Verification items for the finished model (mm, model axes). A direction names the side the tool comes from. Round coordinates to 2 decimals unless told otherwise and drop trailing zeros. Order: outer loops, then holes, each group sorted by start corner. A loop starts at its lowest first (then second) coordinate and runs counter-clockwise, first axis right, second up. Notation, with made-up numbers: (82.5, 20.5) -> (135.5, 20.5) arc R16 ccw to (135.5, 51.5) -> close; hole circle Ø7 at (0, -6.5). An arc over 180 degrees is marked (long way). Answer in a Markdown table with one row per item. Add a question column.
```python
from build123d import *

# Parameters (mm, degrees)
HEX_HEAD_15AF_DEPTH = 8


with BuildPart() as part:
    # Hex Head Profile → Hex Head 15AF (new body)
    with BuildSketch(Plane(origin=(0, 0, 0), x_dir=(1, 0, 0), z_dir=(0, 1, 0))):
        Polygon((8.660254038, 0), (4.330127019, 7.5), (-4.330127019, 7.5), (-8.660254038, 0), (-4.330127019, -7.5), (4.330127019, -7.5), align=None)
    extrude(amount=HEX_HEAD_15AF_DEPTH)

    # Shank Profile → Shank with Cone Point (revolve)
    with BuildSketch(Plane.XY, mode=Mode.PRIVATE) as shank_with_cone_point_sk:
        Polygon((0, 8), (0, 23.886751346), (5, 21), (5, 8), align=None)
    revolve(shank_with_cone_point_sk.sketch.rotate(Axis((0, 23.886751346, 0), (0, 1, 0)), 90), axis=Axis((0, 23.886751346, 0), (0, 1, 0)))

    # Head Chamfer Profile → Head Chamfer Cut (revolve, cut)
    with BuildSketch(Plane.XY, mode=Mode.PRIVATE) as head_chamfer_cut_sk:
        with BuildLine():
            Line((8.660254038, 0), (6.660254038, 0))
            ThreePointArc((6.660254038, 0), (8.0744676, 0.585786438), (8.660254038, 2))
            Line((8.660254038, 2), (8.660254038, 0))
        make_face()
    revolve(head_chamfer_cut_sk.sketch.rotate(Axis((0, 0, 0), (0, 1, 0)), 90), axis=Axis((0, 0, 0), (0, 1, 0)), mode=Mode.SUBTRACT)


solid = part.part
```
1) Cross-section at C-C, the plane y = 21.5. Record the boundary of the cut face in (x, z).
2) Tool access check on faces 1 (the face through (6.526, 4.038, -3.698)), 2 (the face through (2, 8, -5)). Record the directions out of +Z, -Z, +X, -X, +Y, -Y that give a thin tool (end or side, any length) a straight path to the whole face; none if there is none.
3) Cross-section at B-B, the plane y = 17.75. Record the boundary of the cut face in (x, z).
4) Cross-section at A-A, the plane y = 3.75. Record the boundary of the cut face in (x, z).
5) Depth check by flat-ended pin: P1, Ø6, axis at y = 13.5, z = -2, coming from the +X side; P2, Ø4, axis at x = 6.5, z = 0, coming from the +Y side; P3, Ø4, axis at x = 4.5, y = 16, coming from the -Z side. Enter the tip coordinate at first touch or a pass-through.
6) Thickness scan on L1, parallel to X at y = 15.5, z = -0.25; L2, parallel to Y at x = 1.5, z = -6.25; L3, parallel to Y at x = 4.25, z = 1.5. Record the ranges inside material, lowest first. Write a range as [from, to].
Results below:
| question | item | result |
|---|---|---|
| 1 | outline | circle Ø8.27 at (0, 0) |
| 2 | face 1 | -Z, +X, +Y, -Y |
| 2 | face 2 | +Y |
| 3 | outline | circle Ø10 at (0, 0) |
| 4 | outline | (-8.66, 0) -> (-4.33, -7.5) -> (4.33, -7.5) -> (8.66, 0) -> (4.33, 7.5) -> (-4.33, 7.5) -> close |
| 5 | P1 | x = 5 |
| 5 | P2 | y = 21.29 |
| 5 | P3 | z = -4.33 |
| 6 | L1 | [-4.99, 4.99] |
| 6 | L2 | [0, 8] |
| 6 | L3 | [0, 21.28] |
